The drawing under review shows one solid part. Ordinate dimensions are in mm from its lowest x, y, z. Give positions to 0.01 mm unless a question says otherwise; leave off trailing zeros. Loops run counter-clockwise (first coordinate to the right, second up) from the corner with the lowest first, then second, coordinate; pieces in that order, holes last. Notation, with made-up numbers: (-3.75, -32) - (13.25, -32) arc R18 ccw to (13.25, -13) - close; hole circle Ø6 at (25, 69.25). An arc over 180 degrees is marked (long way). Write each question's results on one line, items separated by ' | '.
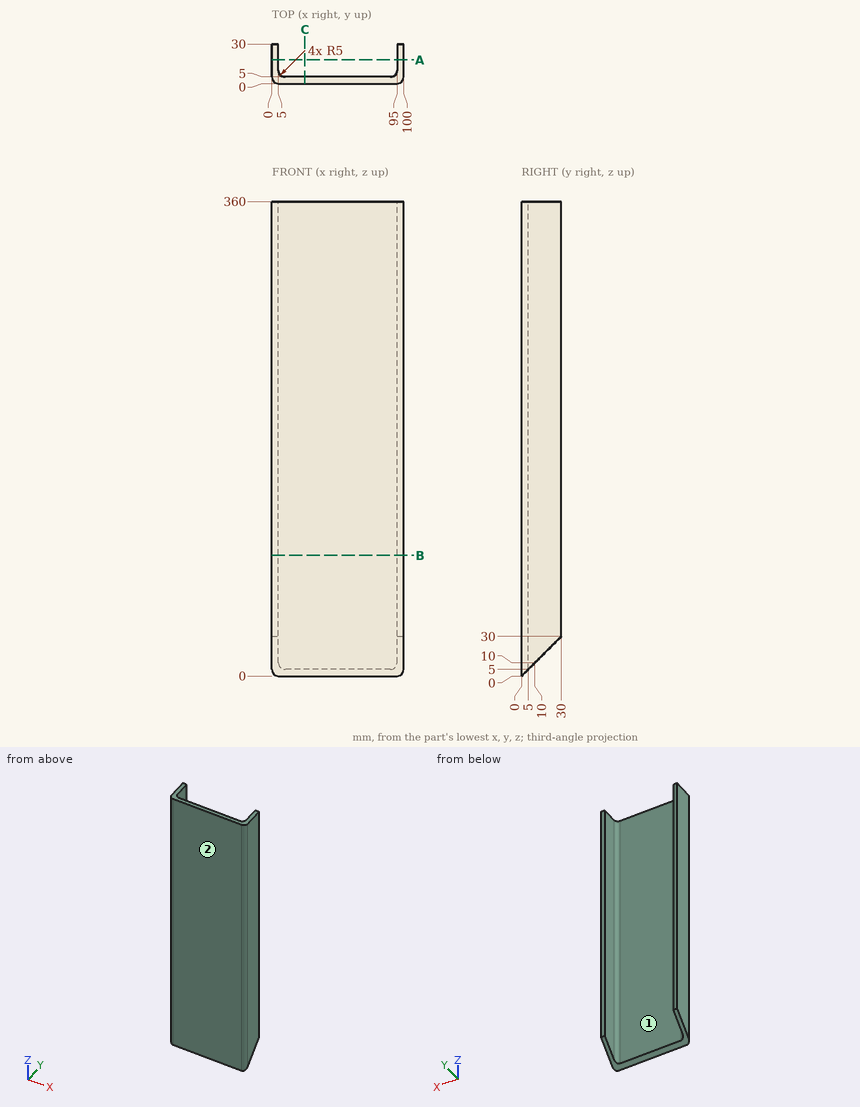
(1) Insertion check: P1, Ø5, axis at x = 45, z = 97, coming from the +Y side. The pin has a flat end and moves straight along its axis. Give the tip position at first contact, or say it passes through.
Answers below:
P1: y = 5
(2) Take a section at C-C on x = 25. Give the boundary of the cut face in (y, z), plus the area to 3 significant figures.
Answers below:
outline: (0, 0) - (5, 5) - (5, 360) - (0, 360) - close | area: 1,790 mm2
(3) Take a section at B-B on z = 91.5. Give the boundary of the cut face in (x, y), plus the area to 3 significant figures.
Answers below:
outline: (0, 5) arc R5 ccw to (5, 0) - (95, 0) arc R5 ccw to (100, 5) - (100, 30) - (95, 30) - (95, 10) arc R5 cw to (90, 5) - (10, 5) arc R5 cw to (5, 10) - (5, 30) - (0, 30) - close | area: 750 mm2
(4) Take a section at A-A on y = 18. Give the boundary of the cut face in (x, z).
Answers below:
outline: (0, 18) - (5, 18) - (5, 360) - (0, 360) - close; (95, 18) - (100, 18) - (100, 360) - (95, 360) - close
(5) Wall thickness on line 1 along X through (y, z) = (10, 32.5); line 2 along Y through (x, z) = (81.5, 142); line 3 along X through (y, z) = (5.5, 165): over which ranges is each line inside the solid? List them lowest first. Write a range as from..to.
Answers below:
line 1: 0..5, 95..100 | line 2: 0..5 | line 3: 0..7.82, 92.18..100
(6) Draft analysis for pull direction X (two halves, no side actions). For the marked faces 1 and 2, state which applies: pulls with the +X half, pulls with the -X half, needs draft (parallel to the pull), parting line crosses it, or undercut.
Answers below:
face 1: undercut | face 2: needs draft
